Verification items for the finished model (mm, model axes). Face numbers are marked on the shaded views. Coordinates: 2 decimals unless noted, no trailing zeros. Write each loop counter-clockwise with the first axis right and the second up, starting at its lowest first coordinate (ties: lowest second). Pieces come first, ordered by that corner, then holes. Notation, with made-up numbers: (-20, -2) -> (37, -2) arc R15 cw to (37, 7) -> close; hole circle Ø10 at (-24.75, -34.5). An arc over 180 degrees is marked (long way). Write each question's results on one line, items separated by ' | '. Start each with the question number.
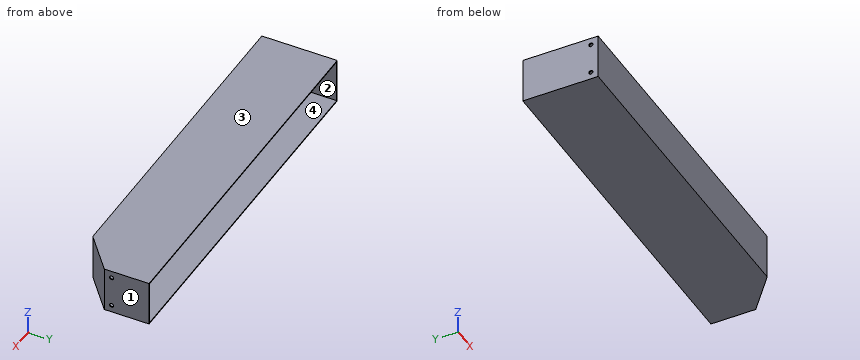
from build123d import *

# Parameters (mm, degrees)
EXTRUDE_1_DEPTH     = 100
SHELL_1_T           = -2
SKETCH_2_R          = 4.5
CUT_EXTRUDE_1_DEPTH = 10
SKETCH_3_R          = 4.5
CUT_EXTRUDE_2_DEPTH = 10


with BuildPart() as part:
    # 草图1 → 凸台-拉伸1 (new body)
    with BuildSketch(Plane.XY):
        Polygon((0, 0), (707.152509296, 0), (787, 67), (787, 165), (0, 165), align=None)
    extrude(amount=EXTRUDE_1_DEPTH)

    # 抽壳1
    shell_1_openings = [part.faces().sort_by_distance(p)[0] for p in [
        (393.5, 165, 50),
    ]]
    offset(amount=SHELL_1_T, openings=shell_1_openings, kind=Kind.INTERSECTION)

    # 草图2 → 切除-拉伸1 (cut)
    with BuildSketch(Plane.ZY):
        with Locations(Location((16, 16, 0), (0, 0, 270))):
            Circle(SKETCH_2_R)
        with Locations(Location((84, 16, 0), (0, 0, 270))):
            Circle(SKETCH_2_R)
    extrude(amount=-CUT_EXTRUDE_1_DEPTH, mode=Mode.SUBTRACT)

    # 草图3 → 切除-拉伸2 (cut)
    with BuildSketch(Plane(origin=(787, 0, 0), x_dir=(0, 0, -1), z_dir=(1, 0, 0))):
        with Locations((-84, 83)):
            Circle(SKETCH_3_R)
        with Locations((-16, 83)):
            Circle(SKETCH_3_R)
    extrude(amount=-CUT_EXTRUDE_2_DEPTH, mode=Mode.SUBTRACT)


solid = part.part
1. Depth check by flat-ended pin: pin 1 Ø5.5 at (y, z) = (16, 84) entering from -X; pin 2 Ø6 at (x, z) = (140.5, 68) entering from +Y; pin 3 Ø10.5 at (y, z) = (16, 16) entering from +X. Enter the tip coordinate at first touch or a pass-through.
2. Sectioned sample at C-C on y = 42.5. Record the cut outline in (x, z).
3. Sectioned sample at A-A on x = 522. Record the cut outline in (y, z), plus the area to 3 significant figures.
4. Sectioned sample at B-B on z = 56.5. Record the cut outline in (x, y).
5. Material ranges on probe 1 along Z at (x, y) = (495.5, 153.5); probe 2 along X at (y, z) = (96.5, 95); probe 3 along Y at (x, z) = (300, 58), recorded low to high. Write a range as from..to.
6. Mould release check, pull along Z, two halves, no side actions. Record for the marked faces 1, 2, 3 and 4: +Z half, -Z half, draft (parallel to the pull), parting line (faces both ways), or undercut.
Computed values:
1) pin 1: stops at x = 719.83 | pin 2: stops at y = 2 | pin 3: stops at x = 732.48
2) outline: (0, 0) -> (757.8, 0) -> (757.8, 100) -> (0, 100) -> close; hole (2, 2) -> (754.69, 2) -> (754.69, 98) -> (2, 98) -> close
3) outline: (0, 0) -> (165, 0) -> (165, 2) -> (2, 2) -> (2, 98) -> (165, 98) -> (165, 100) -> (0, 100) -> close | area: 852 mm^2
4) outline: (0, 0) -> (707.15, 0) -> (787, 67) -> (787, 165) -> (785, 165) -> (785, 67.93) -> (706.42, 2) -> (2, 2) -> (2, 165) -> (0, 165) -> close
5) probe 1: z = 0..2, 98..100 | probe 2: x = 0..2, 785..787 | probe 3: y = 0..2
6) face 1: draft | face 2: undercut | face 3: +Z half | face 4: undercut
